Design review of the part built by this model. Coordinates are the model's own, in mm. Face numbers are marked on the shaded views. A direction names the side the tool comes from. Coordinates: 2 decimals unless noted, no trailing zeros. Loops run counter-clockwise (first coordinate to the right, second up) from the corner with the lowest first, then second, coordinate; pieces in that order, holes last. Notation, with made-up numbers: (89.25, 46) -> (134.25, 46) arc R13 cw to (134.25, 51) -> close; hole circle Ø2 at (-3.75, -0.5). An arc over 180 degrees is marked (long way). Answer in a Markdown table with one row per item.
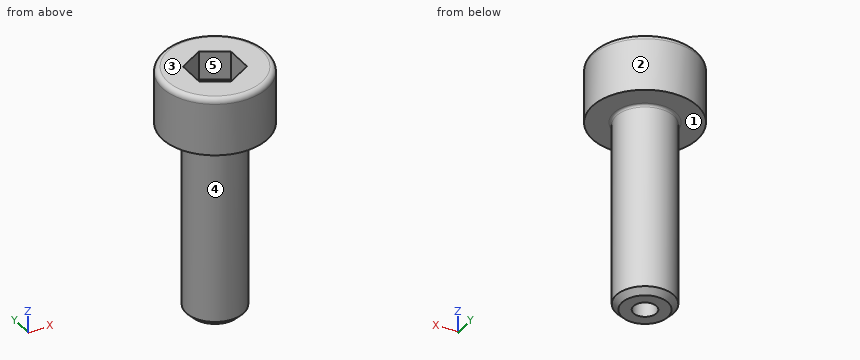
```python
from build123d import *

# Parameters (mm, degrees)
CUT_EXTRUDE1_DEPTH = 1.5
FILLET1_R          = 0.275
CHAMFER1_SIZE      = 0.3
FILLET2_R          = 0.125


with BuildPart() as part:
    # Sketch3 → Revolve1 (revolve)
    with BuildSketch(Plane(origin=(0, 0, 0), x_dir=(0, 0, -1), z_dir=(1, 0, 0)), mode=Mode.PRIVATE) as revolve1_sk:
        Polygon((-3, 0.6), (-3, 2.75), (0, 2.75), (0, 1.5), (10, 1.5), (10, 0.6), align=None)
    revolve(revolve1_sk.sketch.rotate(Axis((0, 0, 3), (0, 0, -1)), 90), axis=Axis((0, 0, 3), (0, 0, -1)))

    # Sketch4 → Cut-Extrude1 (cut)
    with BuildSketch(Plane.XY.offset(3)):
        Polygon((0, 1.443375673), (-1.25, 0.721687836), (-1.25, -0.721687836), (0, -1.443375673), (1.25, -0.721687836), (1.25, 0.721687836), align=None)
    extrude(amount=-CUT_EXTRUDE1_DEPTH, mode=Mode.SUBTRACT)

    # Fillet1
    fillet1_edges = [part.edges().sort_by_distance(p)[0] for p in [
        (-2.75, 0, 3),
    ]]
    fillet(fillet1_edges, radius=FILLET1_R)

    # Chamfer1
    chamfer1_edges = [part.edges().sort_by_distance(p)[0] for p in [
        (-1.5, 0, -10),
    ]]
    chamfer(chamfer1_edges, length=CHAMFER1_SIZE)

    # Cut-Extrude2 cone 1 section (through the dimple's axis) → Cut-Extrude2 (revolve, cut)
    with BuildSketch(Plane(origin=(0, 0, 1.5), x_dir=(0, -1, 0), z_dir=(1, 0, 0))):
        Polygon((0, 0), (1.25, 0), (0, 0.721687836), align=None)
    revolve(axis=Axis((0, 0, 1.5), (0, 0, -1)), mode=Mode.SUBTRACT)

    # Fillet2
    fillet2_edges = [part.edges().sort_by_distance(p)[0] for p in [
        (-1.5, 0, 0),
    ]]
    fillet(fillet2_edges, radius=FILLET2_R)


solid = part.part
```
(1) To check wall thickness, follow probe 1 along Y at (x, z) = (0.05, -5.5); probe 2 along Z at (x, y) = (1.6, -1.6); probe 3 along Y at (x, z) = (0.9, -4.5). State the ranges of each line that lie inside material, in increasing order.
Evaluation:
| item | result |
|---|---|
| probe 1 | y = -1.5 to -0.6, 0.6 to 1.5 |
| probe 2 | z = 0 to 3 |
| probe 3 | y = -1.2 to 1.2 |
(2) For pin 1 (1 mm diameter, centred on x = 1.5, z = -4.5, fed in from -Y); pin 2 (2 mm diameter, centred on y = 0.5, z = -4, fed in from +X), all flat-tipped, find the tip position at first contact; note any pin that passes through.
Evaluation:
| item | result |
|---|---|
| pin 1 | stops at y = -1.12 |
| pin 2 | stops at x = 1.5 |
(3) Draft analysis for pull direction Y (two halves, no side actions). For the marked faces 3, 4 and 5, state which applies: pulls with the +Y half, pulls with the -Y half, needs draft (parallel to the pull), parting line crosses it, or undercut.
Evaluation:
| item | result |
|---|---|
| face 3 | needs draft |
| face 4 | parting line crosses it |
| face 5 | undercut |
(4) Take a section at A-A on z = -6.75. Give the boundary of the cut face in (x, y), and give its area (3 significant figures).
Evaluation:
| item | result |
|---|---|
| outline | circle Ø3 at (0, 0); hole circle Ø1.2 at (0, 0) |
| area | 5.94 mm² |
(5) Tool access review of the marked faces 1 and 2: name each direction out of +Z, -Z, +X, -X, +Y, -Y from which nothing blocks a thin tool from reaching the whole face with its end or side.
Evaluation:
| item | result |
|---|---|
| face 1 | -Z |
| face 2 | +Z, -Z |
